Can you work these out from the model? Positions are in its coordinate system, mm. A direction names the side the tool comes from. Give positions to 0.01 mm unless a question says otherwise; leave off trailing zeros. Order: outer loops, then holes, each group sorted by start corner. A loop starts at its lowest first (then second) coordinate and runs counter-clockwise, first axis right, second up. Notation, with made-up numbers: (89, 47.5) -> (105, 47.5) arc R8 cw to (105, 51.5) -> close; hole circle Ø9 at (76, 44). An arc over 180 degrees is marked (long way). Answer as CSV lines item,"result".
```python
from build123d import *

# Parameters (mm, degrees)
BASE_BLOCK_SKETCH_R              = 40
BASE_BLOCK_SKETCH_R_2            = 20
BASE_BLOCK_40MM_DEPTH            = 20
BRACKET_PLATE_PROFILE_SKETCH_R   = 20
BRACKET_PLATE_PROFILE_SKETCH_R_2 = 8
BRACKET_PLATE_16MM_DEPTH         = 8
BORE_BOSSES_DEPTH                = 15
BORE_BOSSES_DEPTH_BACK           = 45
BORE_BOSSES_START                = 8
SKETCH2_3_R                      = 25


with BuildPart() as part:
    # Base Block Sketch → Base Block 40mm (new, symmetric)
    with BuildSketch(Plane.XY):
        Circle(BASE_BLOCK_SKETCH_R)
        Circle(BASE_BLOCK_SKETCH_R_2, mode=Mode.SUBTRACT)
    extrude(amount=BASE_BLOCK_40MM_DEPTH, both=True)

    # Bracket Plate Profile Sketch → Bracket Plate 16mm (add, symmetric)
    with BuildSketch(Plane.XY):
        with BuildLine():
            ThreePointArc((-38.79460493, 9.74569794), (-31.60581958, -24.516773211), (-0.207064055, -39.999464052))
            Line((-0.207064055, -39.999464052), (129.230816729, -40.669521341))
            ThreePointArc((129.230816729, -40.669521341), (180.148903337, -0.446830099), (152.19937164, 58.1137378))
            Line((152.19937164, 58.1137378), (20.453770296, 122.036129806))
            ThreePointArc((20.453770296, 122.036129806), (-1.027993314, 122.200069977), (-14.706017228, 105.634904541))
            Line((-14.706017228, 105.634904541), (-38.79460493, 9.74569794))
        make_face()
        Circle(BRACKET_PLATE_PROFILE_SKETCH_R, mode=Mode.SUBTRACT)
        Polygon((132.550450996, -23.537032507), (97.683636563, -26.587483503), (94.633185567, 8.27933093), (91.582734571, 43.146145364), (126.449549004, 46.19659636), (161.316363437, 49.247047356), (164.366814433, 14.380232923), (167.417265429, -20.48658151), align=None, mode=Mode.SUBTRACT)
        with Locations((9.540610853, 99.543843328)):
            Circle(BRACKET_PLATE_PROFILE_SKETCH_R_2, mode=Mode.SUBTRACT)
    extrude(amount=BRACKET_PLATE_16MM_DEPTH, both=True)

    # Sketch2_3 → Bore Bosses (add, two sides: drawn at the far end of the back side and taken through both)
    with BuildSketch(Plane.XY.offset(BORE_BOSSES_START - BORE_BOSSES_DEPTH_BACK)):
        Polygon((94.633185567, 8.27933093), (91.582734571, 43.146145364), (126.449549004, 46.19659636), (161.316363437, 49.247047356), (164.366814433, 14.380232923), (167.417265429, -20.48658151), (132.550450996, -23.537032507), (97.683636563, -26.587483503), align=None)
        with Locations((129.5, 11.329781927)):
            Circle(SKETCH2_3_R, mode=Mode.SUBTRACT)
    extrude(amount=BORE_BOSSES_DEPTH + BORE_BOSSES_DEPTH_BACK)


solid = part.part
```
Item 1: For faces 4 (the flat face through (126.94, 46.24, 15.39)), 5 (the flat face through (-9.4, 18.3, 20)), 6 (the flat face through (164.41, 13.89, 15.39)), which set-ups out of +Z, -Z, +X, -X, +Y, -Y let a thin tool reach every point of the face, with its end or its side?
Numbers:
face 4,"+Z, -X, +Y"
face 5,"+Z, -X, +Y, -Y"
face 6,"+Z, +X, +Y"
Item 2: Imagine slicing it at B-B, the plane x = -9. Please give me the cut outline in (y, z), then the cut area to 3 significant figures.
Numbers:
outline,"(-38.97, -20) -> (-17.86, -20) -> (-17.86, 20) -> (-38.97, 20) -> close; (17.86, -20) -> (38.97, -20) -> (38.97, -8) -> (116.31, -8) -> (116.31, 8) -> (38.97, 8) -> (38.97, 20) -> (17.86, 20) -> close"
area,"2,930 mm²"
Item 3: We'd pull the mould along X, two halves only. Please class faces 1 (the cylindrical face through (-0.745, 122.33, 0.112)), 2 (the flat face through (-9.4, 18.3, -20)), 3 (the cylindrical face through (-32, -24, 0)): released by +X, released by -X, zero draft, split by the parting line, or undercut.
Numbers:
face 1,"split by the parting line"
face 2,"zero draft"
face 3,"undercut"
Item 4: Imagine slicing it at D-D, the plane x = 34.5. Please give me the cut outline in (y, z).
Numbers:
outline,"(-40.18, -8) -> (-20.24, -8) -> (-20.24, -20) -> (20.24, -20) -> (20.24, -8) -> (115.22, -8) -> (115.22, 8) -> (20.24, 8) -> (20.24, 20) -> (-20.24, 20) -> (-20.24, 8) -> (-40.18, 8) -> close"
Item 5: For pin 1 (5 mm diameter, centred on x = 127.5, z = 17, fed in from +Y); pin 2 (1 mm diameter, centred on x = 118.5, z = 10.5, fed in from +Y); pin 3 (6 mm diameter, centred on x = 62.5, y = 86.5, fed in from -Z), each with a flat end and sliding along its axis, tell me the tip position at first contact or that it passes through.
Numbers:
pin 1,"stops at y = 46.51"
pin 2,"stops at y = 45.54"
pin 3,"stops at z = -8"
Item 6: Imagine slicing it at C-C, the plane y = 0. Please give me the cut outline in (x, z), then the cut area to 3 significant figures.
Numbers:
outline,"(-40, -20) -> (-20, -20) -> (-20, 20) -> (-40, 20) -> close; (20, -20) -> (40, -20) -> (40, -8) -> (95.36, -8) -> (95.36, -37) -> (107.21, -37) -> (107.21, 23) -> (95.36, 23) -> (95.36, 8) -> (40, 8) -> (40, 20) -> (20, 20) -> close; (151.79, -37) -> (165.62, -37) -> (165.62, -8) -> (180.25, -8) -> (180.25, 8) -> (165.62, 8) -> (165.62, 23) -> (151.79, 23) -> close"
area,"4,260 mm²"
Item 7: Please list where these lines run through material, in increasing order: line 1 along X through (y, z) = (13.5, 0.5); line 2 along Y through (x, z) = (0, 12); line 3 along Z through (x, y) = (76, 44.5).
Numbers:
line 1,"x = -37.85 to -14.76, 14.76 to 104.59, 154.41 to 181.45"
line 2,"y = -40 to -20, 20 to 40"
line 3,"z = -8 to 8"
Item 8: Imagine slicing it at A-A, the plane z = 12. Please give me the cut outline in (x, y), then the cut area to 3 significant figures.
Numbers:
outline,"circle Ø80 at (0, 0); (91.58, 43.15) -> (97.68, -26.59) -> (167.42, -20.49) -> (161.32, 49.25) -> close; hole circle Ø40 at (0, 0); hole circle Ø50 at (129.5, 11.33)"
area,"6,710 mm²"
